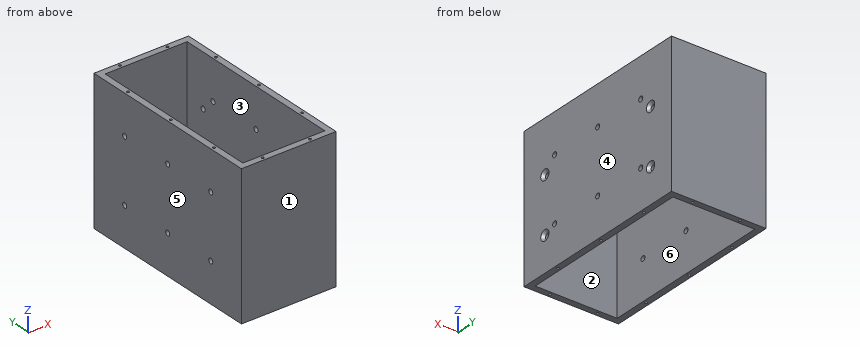
from build123d import *

# Parameters (mm, degrees)
SKETCH_1_W                   = 60
SKETCH_1_H                   = 120
EXTRUDE_1_DEPTH              = 45
SHELL_1_T                    = -4
HOLE_WIZARD_M2_1_D           = 1.6
HOLE_WIZARD_M2_1_DEPTH       = 5.2
HOLE_WIZARD_M2_1_TIP         = 0.480688495
HOLE_WIZARD_M2_2_D           = 1.6
HOLE_WIZARD_M2_2_DEPTH       = 5.2
HOLE_WIZARD_M2_2_TIP         = 0.480688495
HOLE_WIZARD_M3_1_D           = 3.4
HOLE_WIZARD_M3_1_DEPTH       = 4
HOLE_WIZARD_M3_1_CSINK_D     = 6.72
HOLE_WIZARD_M3_1_CSINK_ANGLE = 90
HOLE_WIZARD_M4_1_D           = 3.3


with BuildPart() as part:
    # 草图1 → 凸台-拉伸1 (new, symmetric)
    with BuildSketch(Plane.XY):
        Rectangle(SKETCH_1_W, SKETCH_1_H)
    extrude(amount=EXTRUDE_1_DEPTH, both=True)

    # 抽壳1
    shell_1_openings = [part.faces().sort_by_distance(p)[0] for p in [
        (0, 0, 45),
        (0, 0, -45),
    ]]
    offset(amount=SHELL_1_T, openings=shell_1_openings, kind=Kind.INTERSECTION)

    # M2 螺纹孔1
    with Locations(Plane.XY.offset(45)):
        with Locations((-15, -58), (-28, 0), (28, 0), (-15, 58), (15, 58), (-28, 35), (28, 35), (28, -35), (-28, -35), (15, -58)):
            Hole(HOLE_WIZARD_M2_1_D / 2, depth=HOLE_WIZARD_M2_1_DEPTH)
            with Locations((0, 0, -(HOLE_WIZARD_M2_1_DEPTH + HOLE_WIZARD_M2_1_TIP / 2))):  # 118° drill point
                Cone(0, HOLE_WIZARD_M2_1_D / 2, HOLE_WIZARD_M2_1_TIP, mode=Mode.SUBTRACT)

    # M2 螺纹孔2
    with Locations(Plane(origin=(0, 0, -45), x_dir=(-1, 0, 0), z_dir=(0, 0, -1))):
        with Locations((28, 0), (-28, 0), (-15, 58), (15, 58), (28, 35), (-28, 35), (-28, -35), (28, -35), (-15, -58), (15, -58)):
            Hole(HOLE_WIZARD_M2_2_D / 2, depth=HOLE_WIZARD_M2_2_DEPTH)
            with Locations((0, 0, -(HOLE_WIZARD_M2_2_DEPTH + HOLE_WIZARD_M2_2_TIP / 2))):  # 118° drill point
                Cone(0, HOLE_WIZARD_M2_2_D / 2, HOLE_WIZARD_M2_2_TIP, mode=Mode.SUBTRACT)

    # M3 六角凹锥坑螺钉的锥形沉头孔1
    with Locations(Plane(origin=(30, 0, 0), x_dir=(0, 0, -1), z_dir=(1, 0, 0))):
        with Locations((-12, 43), (23, 43), (-12, -43), (23, -43)):
            CounterSinkHole(HOLE_WIZARD_M3_1_D / 2, HOLE_WIZARD_M3_1_CSINK_D / 2, depth=HOLE_WIZARD_M3_1_DEPTH, counter_sink_angle=HOLE_WIZARD_M3_1_CSINK_ANGLE)

    # M4 螺纹孔1 (through all)
    with Locations(Plane(origin=(30, 0, 0), x_dir=(0, 0, -1), z_dir=(1, 0, 0))):
        with Locations((20, 35), (-20, -35), (-20, 35), (20, -35), (-20, 0), (20, 0)):
            Hole(HOLE_WIZARD_M4_1_D / 2)


solid = part.part
For this review, take the finished solid that the model builds, in its own axes (mm). Face numbers are marked on the shaded views. A direction names the side the tool comes from. Coordinates: 2 decimals unless noted, no trailing zeros. Order: outer loops, then holes, each group sorted by start corner. A loop starts at its lowest first (then second) coordinate and runs counter-clockwise, first axis right, second up. Notation, with made-up numbers: (30, 87.5) - (52, 87.5) arc R21 cw to (52, 106.5) - close; hole circle Ø8 at (47.5, 67.25). An arc over 180 degrees is marked (long way). Answer as CSV lines item,"result". Start each with the question number.
1) Add section B-B (z = -23). State the section outline as (x, y) points.
2) Machinability: for the marked faces 5 and 6, which of the approach directions +Z, -Z, +X, -X, +Y, -Y give a long, thin tool a straight path to every point of the face, cutting with its end or side? Answer none if there is none.
3) Add section D-D (z = 34). State the section outline as (x, y) points, then the cut area to 3 significant figures.
4) Draft analysis for pull direction Y (two halves, no side actions). For the marked faces 1, 2, 3 and 4, state which applies: +Y half, -Y half, draft (parallel to the pull), parting line (faces both ways), or undercut.
5) Add section A-A (y = 22.5). State the section outline as (x, z) points, then the cut area to 3 significant figures.
6) Add section C-C (x = 21). State the section outline as (y, z) points, then the cut area to 3 significant figures.
7) To check wall thickness, follow line 1 along Z through (x, y) = (27, 43); line 2 along Y through (x, z) = (15, 41.55); line 3 along Y through (x, z) = (28, -42.4). State the ranges of each line that lie inside material, in increasing order. Write a range as [from, to].
8) Insertion check: P1, Ø2, axis at y = -35, z = -20, coming from the +X side; P2, Ø1.4, axis at x = -28, y = 35, coming from the +Z side. Each pin has a flat end and moves straight along its axis. Give the tip position at first contact, or say it passes through.
Result:
1,outline,"(-30, -60) - (30, -60) - (30, -46.36) - (28.34, -44.7) - (26, -44.7) - (26, -56) - (-26, -56) - (-26, 56) - (26, 56) - (26, 44.7) - (28.34, 44.7) - (30, 46.36) - (30, 60) - (-30, 60) - close; (26, -41.3) - (28.34, -41.3) - (30, -39.64) - (30, 39.64) - (28.34, 41.3) - (26, 41.3) - close"
2,face 5,"+Z, -Z, -X, +Y, -Y"
2,face 6,"+Z, -Z"
3,outline,"(-30, -60) - (30, -60) - (30, 60) - (-30, 60) - close; hole (-26, -56) - (26, -56) - (26, 56) - (-26, 56) - close"
3,area,"1,380 mm^2"
4,face 1,"-Y half"
4,face 2,"undercut"
4,face 3,"undercut"
4,face 4,"draft"
5,outline,"(-30, -45) - (-26, -45) - (-26, 45) - (-30, 45) - close; (26, -45) - (30, -45) - (30, 45) - (26, 45) - close"
5,area,"720 mm^2"
6,outline,"(-60, -45) - (-56, -45) - (-56, 45) - (-60, 45) - close; (56, -45) - (60, -45) - (60, 45) - (56, 45) - close"
6,area,"720 mm^2"
7,line 1,"[-45, -24.7], [-21.3, 10.3], [13.7, 45]"
7,line 2,"[-60, -58.8], [-57.2, -56], [56, 57.2], [58.8, 60]"
7,line 3,"[-60, -35.8], [-34.2, -0.8], [0.8, 34.2], [35.8, 60]"
8,P1,"through"
8,P2,"z = 39.74"
